```python
from build123d import *

# Parameters (mm, degrees)
BOSS_EXTRUDE2_DEPTH = 2.5


with BuildPart() as part:
    # Sketch1 → Revolve1 (revolve)
    with BuildSketch(Plane(origin=(0, 0, 0), x_dir=(0, 0, -1), z_dir=(1, 0, 0))):
        Polygon((253, -0.618600266), (253, 1.381399734), (99.973878508, 9.381399734), (0, 9.381399734), (0, 10.381399734), (100, 10.381399734), (254, 2.330486674), (254, 1.381399734), (254, -0.618600266), align=None)
    revolve(axis=Axis((0, 0, 0), (0, 1, 0)))

    # Sketch2 → Boss-Extrude2 (add, symmetric)
    with BuildSketch(Plane(origin=(0, 0, 0), x_dir=(0, 0, -1), z_dir=(1, 0, 0))):
        Polygon((-48, 10.381399734), (-48, 35.381399734), (48, 35.381399734), (48, 10.381399734), (50, 10.381399734), (50, 40.381399734), (-50, 40.381399734), (-50, 10.381399734), align=None)
    extrude(amount=BOSS_EXTRUDE2_DEPTH, both=True)


solid = part.part
```
Verification items for the finished model (mm, model axes). A direction names the side the tool comes from. Give positions to 0.01 mm unless a question says otherwise; leave off trailing zeros. Order: outer loops, then holes, each group sorted by start corner. A loop starts at its lowest first (then second) coordinate and runs counter-clockwise, first axis right, second up. Notation, with made-up numbers: M -10,14.25 L 45,14.25 A23 cw 45,51.25 Z; hole C -24,-3.75 d7. An arc over 180 degrees is marked long. Answer in a Markdown table with one row per item. Add a question column.
Item 1: Tool access check on faces 4 (the cylindrical face through (247.96, 0.88, 55.06)), 5 (the flat face through (-1, 9.381, 1)), 6 (the flat face through (2.5, 37, 8)). Record the directions out of +Z, -Z, +X, -X, +Y, -Y that give a thin tool (end or side, any length) a straight path to the whole face; none if there is none.
Item 2: Mould release check, pull along Z, two halves, no side actions. Record for faces 1 (the flat face through (-2.5, 37, 8)), 2 (the cylindrical face through (-250.847, 0.395, 32.936)), 3 (the conical face through (-32.931, 9.878, -104.571)): released by +Z, released by -Z, zero draft, split by the parting line, or undercut.
Item 3: Scan lines: probe 1 along Z at (x, y) = (0, -0.05); probe 2 along Y at (x, z) = (-219, -121). Record each from-to range of solid material in increasing order. Write a range as from..to.
Item 4: Gauge pin test, flat ends, axial feed: pin 1 (4 mm diameter, centred on x = 0.5, y = 28.5, fed in from +Z); pin 2 (1 mm diameter, centred on y = 11, z = -56, fed in from -X); pin 3 (2.5 mm diameter, centred on x = 1, y = 23.5, fed in from -Z); pin 4 (5.5 mm diameter, centred on x = -0.5, z = -10, fed in from -Y). Record the tip position at first contact, or that the pin passes through.
Item 5: Section check B-B, the plane y = 28. Enter the section's corners in (x, z), and give its area (3 significant figures).
Item 6: Section check A-A, the plane z = 0. Enter the section's corners in (x, y), and give its area (3 significant figures).
Filled sheet:
| question | item | result |
|---|---|---|
| 1 | face 4 | +Y, -Y |
| 1 | face 5 | -Y |
| 1 | face 6 | +Z, -Z, +X, +Y |
| 2 | face 1 | zero draft |
| 2 | face 2 | undercut |
| 2 | face 3 | split by the parting line |
| 3 | probe 1 | z = -254..-253, 253..254 |
| 3 | probe 2 | y = 1.53..2.53 |
| 4 | pin 1 | stops at z = 50 |
| 4 | pin 2 | passes through |
| 4 | pin 3 | stops at z = -50 |
| 4 | pin 4 | stops at y = 9.38 |
| 5 | outline | M -2.5,-50 L 2.5,-50 L 2.5,-48 L -2.5,-48 Z; M -2.5,48 L 2.5,48 L 2.5,50 L -2.5,50 Z |
| 5 | area | 20.0 mm^2 |
| 6 | outline | M -254,-0.62 L -253,-0.62 L -253,1.38 L -99.97,9.38 L 99.97,9.38 L 253,1.38 L 253,-0.62 L 254,-0.62 L 254,2.33 L 100,10.38 L -100,10.38 L -254,2.33 Z; M -2.5,35.38 L 2.5,35.38 L 2.5,40.38 L -2.5,40.38 Z |
| 6 | area | 537 mm^2 |
